Read the model definition and answer for the solid it produces. Units are mm, in the model's axes. A direction names the side the tool comes from. Give positions to 0.01 mm unless a question says otherwise; leave off trailing zeros. Order: outer loops, then holes, each group sorted by start corner. A loop starts at its lowest first (then second) coordinate and runs counter-clockwise, first axis right, second up.
```python
from build123d import *

# Parameters (mm, degrees)
SKETCH_1_W               = 30
SKETCH_1_H               = 30
EXTRUDE_1_DEPTH          = 20
FILLET_1_R               = 4.5
SKETCH_2_W               = 8.2
SKETCH_2_H               = 0.3
SKETCH_2_H_2             = 1.9
SKETCH_2_R               = 3.4
CUT_EXTRUDE_1_DEPTH      = 46.276925691
PATTERN_CIRCULAR_1_COUNT = 4


with BuildPart() as part:
    # 草图1 → 凸台-拉伸1 (new, symmetric)
    with BuildSketch(Plane.XY):
        Rectangle(SKETCH_1_W, SKETCH_1_H)
    extrude(amount=EXTRUDE_1_DEPTH, both=True)

    # 圆角1
    fillet_1_edges = [part.edges().sort_by_distance(p)[0] for p in [
        (-15, 15, 0),
        (15, 15, 0),
        (15, -15, 0),
        (-15, -15, 0),
    ]]
    fillet(fillet_1_edges, radius=FILLET_1_R)

    # 草图2 → 切除-拉伸1 (cut, through all)
    with BuildSketch(Plane.XY.offset(20)):
        with Locations((0, 12.95)):
            Rectangle(SKETCH_2_W, SKETCH_2_H)
        with Locations((0, 14.05)):
            Rectangle(SKETCH_2_W, SKETCH_2_H_2)
        Polygon((10.25, 13.1), (4.1, 13.1), (4.1, 12.8), (-4.1, 12.8), (-4.1, 13.1), (-10.25, 13.1), (-10.25, 12.5), (-8.429704265, 12.5), (8.429704265, 12.5), (10.25, 12.5), align=None)
        Polygon((3.479704265, 5.3), (8.429704265, 12.5), (-8.429704265, 12.5), (-3.479704265, 5.3), align=None)
        Circle(SKETCH_2_R)
    cut_extrude_1 = extrude(amount=-CUT_EXTRUDE_1_DEPTH, mode=Mode.SUBTRACT)

    # 阵列(圆周)1: 切除-拉伸1 ×4 about axis
    pattern_circular_1_axis = Axis((0, 0, 0), (0, 0, 1))
    for i in range(1, PATTERN_CIRCULAR_1_COUNT):
        add(cut_extrude_1.rotate(pattern_circular_1_axis, i * 360 / PATTERN_CIRCULAR_1_COUNT), mode=Mode.SUBTRACT)


solid = part.part
```
1) The part is cut by section C-C on y = -7.5. Determine the outline of the cut face in (x, z), and give its area (3 significant figures).
Final values:
outline: (-15, -20) - (-13.1, -20) - (-13.1, 20) - (-15, 20) - close; (-11.15, -20) - (-4.99, -20) - (-4.99, 20) - (-11.15, 20) - close; (4.99, -20) - (11.15, -20) - (11.15, 20) - (4.99, 20) - close; (13.1, -20) - (15, -20) - (15, 20) - (13.1, 20) - close
area: 644 mm2
2) Given pin 1 (0.7 mm diameter, centred on y = -13, z = 6.5, fed in from -X); pin 2 (2 mm diameter, centred on x = -14, z = 5, fed in from +Y); pin 3 (1 mm diameter, centred on x = -9.5, y = -4, fed in from +Z); pin 4 (4 mm diameter, centred on x = 2.5, z = -15.5, fed in from -Y), each flat-ended and moving along its own axis, determine where each tip first touches the part or whether it passes through.
Final values:
pin 1: stops at x = -14.45
pin 2: stops at y = 14.24
pin 3: passes through
pin 4: stops at y = -15
3) Consider L1, parallel to Y at x = 0, z = 0.5; L2, parallel to Y at x = 9.5, z = 11. Determine where each line is inside the solid, lowest interval first.
Final values:
L1: y = -5.3 to -3.4, 3.4 to 5.3
L2: y = -15 to -13.1, -12.5 to -6.37, 6.37 to 12.5, 13.1 to 15
4) The part is cut by section A-A on y = 0. Determine the outline of the cut face in (x, z), and give its area (3 significant figures).
Final values:
outline: (-5.3, -20) - (-3.4, -20) - (-3.4, 20) - (-5.3, 20) - close; (3.4, -20) - (5.3, -20) - (5.3, 20) - (3.4, 20) - close
area: 152 mm2
5) For a pull along Y with two mould halves and no side action, classify faces 1 (the face through (13.717, 13.647, -0.28)), 2 (the face through (-12.5, -9, 0)), 3 (the face through (4.1, 14, 0)) as released by +Y, released by -Y, zero draft, split by the parting line, or undercut.
Final values:
face 1: released by +Y
face 2: undercut
face 3: zero draft
6) A tool of negligible diameter and unlimited length cuts with its end or side. For faces 4 (the face through (-5.92, -8.85, 0.28)), 5 (the face through (0, 4, 20)), 6 (the face through (-4.1, -14, 0)), 7 (the face through (-15, -7, 0)), 8 (the face through (-5.3, 0, 0)), from which of +Z, -Z, +X, -X, +Y, -Y can it reach the whole face along a straight path? Write none if from no direction.
Final values:
face 4: +Z, -Z
face 5: +Z, +X, -X, +Y, -Y
face 6: +Z, -Z, -Y
face 7: +Z, -Z, -X, +Y, -Y
face 8: +Z, -Z, -X
